Part model, mm, in its own coordinate system. A direction names the side the tool comes from. Round coordinates to 2 decimals unless told otherwise and drop trailing zeros. Loops run counter-clockwise (first coordinate to the right, second up) from the corner with the lowest first, then second, coordinate; pieces in that order, holes last.
(1) Cut at D-D on x = -3. List the corners of the cut face in (y, z).
(2) Cut at A-A on y = 4.3. List the corners of the cut face in (x, z), then the cut area to 3 significant figures.
(3) Tool access for faces 5 (the face through (2, 0.7, 9)), 6 (the face through (2, 0.7, -9)), 7 (the face through (0, 5.7, 0)): list every direction of +Z, -Z, +X, -X, +Y, -Y with a clear straight run to the whole face (end or side of a thin tool).
(4) Cut at B-B on x = 0. List the corners of the cut face in (y, z).
(5) Mould opens along Z. For faces 1 (the face through (0, 3, -12.5)), 2 (the face through (0.29, 3.16, 5.27)), 3 (the face through (-5, 3, 10)), 4 (the face through (-7.5, 3, 0)) say: +Z half, -Z half, draft (parallel to the pull), parting line (faces both ways), or undercut.
(6) Cut at C-C on z = -7.25. List the corners of the cut face in (x, y).
(7) Flat gauge pins, fed straight in: pin 1 (2.5 mm diameter, centred on x = 0.5, z = -8, fed in from -Y); pin 2 (3 mm diameter, centred on x = 3.5, y = 2.5, fed in from +Z); pin 3 (6 mm diameter, centred on x = 0, z = -7.5, fed in from -Y). Where does each tip first touch, or does it go through?
(8) Probe probe 1 along Z at (x, y) = (0, 4.6); probe 2 along Z at (x, y) = (1.25, 1.2); probe 3 along Z at (x, y) = (-5, 0.3). List the from-to ranges inside material, lowest first.
from build123d import *

# Parameters (mm, degrees)
SKETCH1_W                  = 15
SKETCH1_H                  = 25
BOSS_EXTRUDE1_DEPTH        = 5.7
SKETCH2_W                  = 15
SKETCH2_H                  = 8.5
CUT_EXTRUDE1_DEPTH         = 0.7
CHAMFER1_SIZE              = 5
F_4_5_4_5_DIAMETER_HOLE1_D = 4.5


with BuildPart() as part:
    # Sketch1 → Boss-Extrude1 (new body)
    with BuildSketch(Plane(origin=(0, 0, 0), x_dir=(1, 0, 0), z_dir=(0, 1, 0))):
        Rectangle(SKETCH1_W, SKETCH1_H)
    extrude(amount=BOSS_EXTRUDE1_DEPTH)

    # Sketch2 → Cut-Extrude1 (cut)
    with BuildSketch(Plane.XZ):
        with Locations((0, -8.25)):
            Rectangle(SKETCH2_W, SKETCH2_H)
        with Locations((0, 8.25)):
            Rectangle(SKETCH2_W, SKETCH2_H)
    extrude(amount=-CUT_EXTRUDE1_DEPTH, mode=Mode.SUBTRACT)

    # Chamfer1
    chamfer1_edges = [part.edges().sort_by_distance(p)[0] for p in [
        (7.5, 3.2, 12.5),
        (-7.5, 3.2, 12.5),
        (-7.5, 3.2, -12.5),
        (7.5, 3.2, -12.5),
    ]]
    chamfer(chamfer1_edges, length=CHAMFER1_SIZE)

    # Ø4.5 (4.5) Diameter Hole1 (through all)
    with Locations(Plane(origin=(0, 5.7, 0), x_dir=(1, 0, 0), z_dir=(0, 1, 0))):
        with Locations((0, 7.5), (0, -7.5)):
            Hole(F_4_5_4_5_DIAMETER_HOLE1_D / 2)


solid = part.part
Final values:
1. outline: (0, -4) - (0.7, -4) - (0.7, -12) - (5.7, -12) - (5.7, 12) - (0.7, 12) - (0.7, 4) - (0, 4) - close
2. outline: (-7.5, -7.5) - (-2.5, -12.5) - (2.5, -12.5) - (7.5, -7.5) - (7.5, 7.5) - (2.5, 12.5) - (-2.5, 12.5) - (-7.5, 7.5) - close; hole circle Ø4.5 at (0, -7.5); hole circle Ø4.5 at (0, 7.5)
2. area: 293 mm2
3. face 5: +Z, +X, -X, -Y
3. face 6: -Z, +X, -X, -Y
3. face 7: +Z, -Z, +X, -X, +Y
4. outline: (0, -4) - (0.7, -4) - (0.7, -5.25) - (5.7, -5.25) - (5.7, 5.25) - (0.7, 5.25) - (0.7, 4) - (0, 4) - close; (0.7, -12.5) - (5.7, -12.5) - (5.7, -9.75) - (0.7, -9.75) - close; (0.7, 9.75) - (5.7, 9.75) - (5.7, 12.5) - (0.7, 12.5) - close
5. face 1: -Z half
5. face 2: undercut
5. face 3: +Z half
5. face 4: draft
6. outline: (-7.5, 0.7) - (-2.24, 0.7) - (-2.24, 5.7) - (-7.5, 5.7) - close; (2.24, 0.7) - (7.5, 0.7) - (7.5, 5.7) - (2.24, 5.7) - close
7. pin 1: passes through
7. pin 2: stops at z = 12.5
7. pin 3: stops at y = 0.7
8. probe 1: z = -12.5 to -9.75, -5.25 to 5.25, 9.75 to 12.5
8. probe 2: z = -12.5 to -9.37, -5.63 to 5.63, 9.37 to 12.5
8. probe 3: z = -4 to 4
